from build123d import *

# Parameters (mm, degrees)
LINK_PLATE_15MM_DEPTH        = 15
SLOT_CUT_DEPTH               = 136.462171841
THROUGH_HOLE_PROFILE_R       = 7.5
THROUGH_HOLE_CUT_DEPTH       = 15
PIVOT_BOSS_PROFILE_40_20_R   = 20
PIVOT_BOSS_PROFILE_40_20_R_2 = 10
PIVOT_BOSS_40_DEPTH          = 20


with BuildPart() as part:
    # Link Plate Profile → Link Plate 15mm (new body)
    with BuildSketch(Plane(origin=(0, 0, 0), x_dir=(1, 0, 0), z_dir=(0, 1, 0))):
        with BuildLine():
            Line((114.015316087, 32.376914511), (104.507658043, -3.811542745))
            ThreePointArc((104.507658043, -3.811542745), (99.16042736, -11.877986807), (90, -15))
            Line((90, -15), (0, -15))
            ThreePointArc((0, -15), (-15, 0), (0, 15))
            ThreePointArc((0, 15), (34.323603484, 25.136249162), (57.634146341, 52.292682927))
            ThreePointArc((57.634146341, 52.292682927), (94.991978757, 68.287105906), (114.015316087, 32.376914511))
        make_face()
    extrude(amount=LINK_PLATE_15MM_DEPTH)

    # Slot Profile → Slot Cut (cut, through all)
    with BuildSketch(Plane(origin=(0, 15, 0), x_dir=(1, 0, 0), z_dir=(0, 1, 0))):
        with BuildLine():
            Line((0, 6), (40, 6))
            ThreePointArc((40, 6), (46, 0), (40, -6))
            Line((40, -6), (0, -6))
            ThreePointArc((0, -6), (-6, 0), (0, 6))
        make_face()
    extrude(amount=-SLOT_CUT_DEPTH, mode=Mode.SUBTRACT)

    # Through Hole Profile → Through Hole Cut (cut)
    with BuildSketch(Plane(origin=(0, 15, 0), x_dir=(1, 0, 0), z_dir=(0, 1, 0))):
        with Locations(Location((90, 0, 0), (0, 0, 270))):
            Circle(THROUGH_HOLE_PROFILE_R)
    extrude(amount=-THROUGH_HOLE_CUT_DEPTH, mode=Mode.SUBTRACT)

    # Pivot Boss Profile Ø40-Ø20 → Pivot Boss Ø40 (add)
    with BuildSketch(Plane(origin=(0, 15, 0), x_dir=(1, 0, 0), z_dir=(0, 1, 0))):
        with Locations(Location((85, 40, 0), (0, 0, 270))):
            Circle(PIVOT_BOSS_PROFILE_40_20_R)
        with Locations(Location((85, 40, 0), (0, 0, 270))):
            Circle(PIVOT_BOSS_PROFILE_40_20_R_2, mode=Mode.SUBTRACT)
    extrude(amount=PIVOT_BOSS_40_DEPTH)


solid = part.part
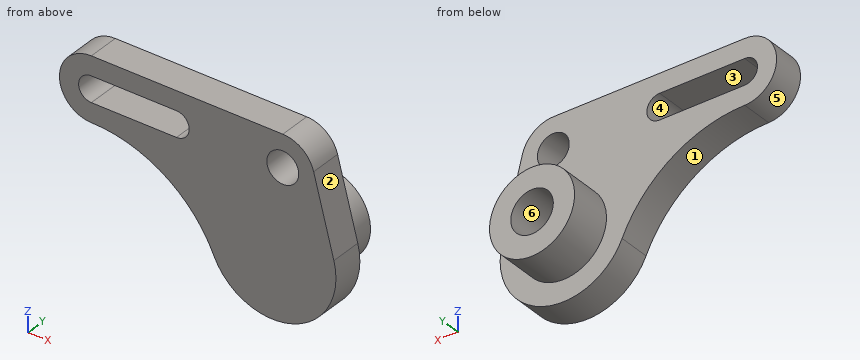
The model under review builds one solid part; all positions refer to its coordinate system, in mm. Face numbers are marked on the shaded views. A direction names the side the tool comes from. Give positions to 0.01 mm unless a question says otherwise; leave off trailing zeros. Order: outer loops, then holes, each group sorted by start corner. A loop starts at its lowest first (then second) coordinate and runs counter-clockwise, first axis right, second up. Notation, with made-up numbers: M 76.5,80 L 83.5,80 A21 ccw 83.5,96 Z; hole C 44,2 d1. An arc over 180 degrees is marked long. Use one line per item in the form item = value. Start each with the question number.
Item 1: We need section D-D on z = -36.5. Give the boundary of the cut face in (x, y).
Item 2: We need section A-A on y = 13. Give the boundary of the cut face in (x, z), plus the area to 3 significant figures.
Item 3: We need section B-B on x = 9. Give the boundary of the cut face in (y, z).
Item 4: To check wall thickness, follow line 1 along X through (y, z) = (8.25, 0); line 2 along Y through (x, z) = (18, -12); line 3 along Z through (x, y) = (44.5, 8). State the ranges of each line that lie inside material, in increasing order. Write a range as from..to.
Item 5: For the marked faces 4, 5 and 6, list the 3-axis set-ups (+Z, -Z, +X, -X, +Y, -Y) from which the entire face can be reached by the end or side of a thin tool; tool diameter is ignored.
Item 6: The part is to be moulded in two halves that separate along Z. For the marked faces 1, 2 and 3, say which applies: pulls with the +Z half, pulls with the -Z half, needs draft (parallel to the pull), parting line crosses it, or undercut.
Item 7: We need section C-C on z = -4. Give the boundary of the cut face in (x, y).
Item 8: Insertion check: pin 1 Ø4 at (y, z) = (16.5, 3) entering from -X; pin 2 Ø4.5 at (x, y) = (11, 10) entering from -Z; pin 3 Ø22 at (x, z) = (83.5, -37) entering from +Y; pin 4 Ø6 at (y, z) = (5, -14) entering from +X. Each pin has a flat end and moves straight along its axis. Give the tip position at first contact, or say it passes through.
Completed:
q1.outline = M 47.48,0 L 114.8,0 L 114.8,15 L 104.69,15 L 104.69,35 L 94.37,35 L 94.37,15 L 75.63,15 L 75.63,35 L 65.31,35 L 65.31,15 L 47.48,15 Z
q2.outline = M 0,-15 A63.18 cw 57.63,-52.29 A30 ccw 114.02,-32.38 L 104.51,3.81 A15 ccw 90,15 L 0,15 A15 ccw Z; hole M 0,-6 L 40,-6 A6 ccw 40,6 L 0,6 A6 ccw Z; hole C 90,0 d15
q2.area = 6,090 mm²
q3.outline = M 0,-15.64 L 15,-15.64 L 15,-6 L 0,-6 Z; M 0,6 L 15,6 L 15,15 L 0,15 Z
q4.line_1 = -15..-6, 46..82.5, 97.5..105.51
q4.line_2 = 0..15
q4.line_3 = -33.33..-3.97, 3.97..15
q5.face_4 = +Y, -Y
q5.face_5 = -X, +Y, -Y
q5.face_6 = +Y
q6.face_1 = pulls with the -Z half
q6.face_2 = pulls with the +Z half
q6.face_3 = undercut
q7.outline = M -14.46,0 L -4.47,0 L -4.47,15 L -14.46,15 Z; M 44.47,0 L 83.66,0 L 83.66,15 L 44.47,15 Z; M 96.34,0 L 106.56,0 L 106.56,15 L 96.34,15 Z
q8.pin_1 = -14.91
q8.pin_2 = -16.4
q8.pin_3 = 35
q8.pin_4 = 109.98
